```python
from build123d import *

# Parameters (mm, degrees)
SKETCH_1_W                  = 130
SKETCH_1_H                  = 600
EXTRUDE_1_DEPTH             = 10
HOLE_WIZARD_2_D             = 6.6
HOLE_WIZARD_2_CBORE_D       = 11
HOLE_WIZARD_2_CBORE_DEPTH   = 6.8
HOLE_WIZARD_M4_2_D          = 3.3
HOLE_WIZARD_2_2_D           = 4.5
HOLE_WIZARD_2_2_CBORE_D     = 8
HOLE_WIZARD_2_2_CBORE_DEPTH = 4.6


with BuildPart() as part:
    # 草图1 → 凸台-拉伸1 (new body)
    with BuildSketch(Plane.XY):
        Rectangle(SKETCH_1_W, SKETCH_1_H)
    extrude(amount=EXTRUDE_1_DEPTH)

    # Hole Wizard 2 (through all)
    with Locations(Plane.XY.offset(10)):
        with Locations((-50, 285), (-50, 0), (-50, -285), (40, 285), (40, -285)):
            CounterBoreHole(HOLE_WIZARD_2_D / 2, HOLE_WIZARD_2_CBORE_D / 2, HOLE_WIZARD_2_CBORE_DEPTH)

    # M4 螺纹孔2 (through all)
    with Locations(Plane.XY.offset(10)):
        with Locations((-56.75, 194), (-56.75, -194)):
            Hole(HOLE_WIZARD_M4_2_D / 2)

    # Hole Wizard 2 2 (through all)
    with Locations(Plane(origin=(0, 0, 0), x_dir=(-1, 0, 0), z_dir=(0, 0, -1))):
        with Locations((-59, -262), (-59, -92), (-59, 92), (-59, 262)):
            CounterBoreHole(HOLE_WIZARD_2_2_D / 2, HOLE_WIZARD_2_2_CBORE_D / 2, HOLE_WIZARD_2_2_CBORE_DEPTH)


solid = part.part
```
Geometry check sheet. Reference: the model listing, model coordinates, mm. A direction names the side the tool comes from. Coordinates: 2 decimals unless noted, no trailing zeros. Answer as a JSON object with one key per item and string values.
Q1. Release check for a two-part mould opening along X. For faces 3 (the flat face through (-1, 300, 5)), 4 (the cylindrical face through (-51.19, -290.37, 6.65)), 5 (the flat face through (44, -285, 3.2)), 6 (the flat face through (-65, -4, 5)) record: released by +X, released by -X, zero draft, split by the parting line, or undercut.
Results are:
{"face 3": "zero draft", "face 4": "undercut", "face 5": "undercut", "face 6": "released by -X"}
Q2. Tool access check on faces 1 (the flat face through (-1, 4, 0)), 2 (the flat face through (-46, 0, 3.2)). Record the directions out of +Z, -Z, +X, -X, +Y, -Y that give a thin tool (end or side, any length) a straight path to the whole face; none if there is none.
Results are:
{"face 1": "-Z, +X, -X, +Y, -Y", "face 2": "+Z"}
Q3. Depth check by flat-ended pin: pin 1 Ø7.5 at (x, y) = (-50, -285) entering from +Z; pin 2 Ø3.5 at (x, y) = (59, 262) entering from -Z; pin 3 Ø6 at (x, y) = (59, -262) entering from -Z. Enter the tip coordinate at first touch or a pass-through.
Results are:
{"pin 1": "stops at z = 3.2", "pin 2": "passes through", "pin 3": "stops at z = 4.6"}
Q4. Scan lines: line 1 (Y direction, x = 59, z = 1.85); line 2 (X direction, y = 285, z = 0.8); line 3 (Y direction, x = -50, z = 8.75). Record each from-to range of solid material in increasing order.
Results are:
{"line 1": "y = -300 to -266, -258 to -96, -88 to 88, 96 to 258, 266 to 300", "line 2": "x = -65 to -53.3, -46.7 to 36.7, 43.3 to 65", "line 3": "y = -300 to -290.5, -279.5 to -5.5, 5.5 to 279.5, 290.5 to 300"}
